Model file for the job. Use its own axes, mm. Face numbers are marked on the shaded views. A direction names the side the tool comes from. Coordinates: 2 decimals unless noted, no trailing zeros. Order: outer loops, then holes, each group sorted by start corner. A loop starts at its lowest first (then second) coordinate and runs counter-clockwise, first axis right, second up. Notation, with made-up numbers: (-14.5, 56.25) -> (35.5, 56.25) arc R19 ccw to (35.5, 72.25) -> close; hole circle Ø6 at (15, 29.5). An arc over 180 degrees is marked (long way). Return JSON: item names as keys, results as strings. Group by question number.
1) Cut at A-A (x = 0). Write the cut outline in (y, z), and give its area (3 significant figures).
2) Pull direction Y, two halves, no side cores. Call the marked faces 3 and 4: +Y half, -Y half, draft (parallel to the pull), parting line (faces both ways), or undercut.
3) Probe line 1 (Y direction, x = 0, z = 2.75); line 2 (Y direction, x = 0, z = 7.2); line 3 (X direction, y = -3.5, z = -7). List the from-to ranges inside material, lowest first.
4) Cut at C-C (z = -5). Write the cut outline in (x, y), and give its area (3 significant figures).
5) Which spindle directions (+Z, -Z, +X, -X, +Y, -Y) get a long thin tool onto all of the face, cutting with end or side? Do the marked faces 1 and 2. Say none if no direction does.
6) Flat gauge pins, fed straight in: pin 1 (4 mm diameter, centred on y = -4, z = -5.5, fed in from -X); pin 2 (1.5 mm diameter, centred on y = 3.5, z = 2.5, fed in from -X). Where does each tip first touch, or does it go through?
from build123d import *

# Parameters (mm, degrees)
SKETCH1_R           = 6
SKETCH1_R_2         = 4
BOSS_EXTRUDE1_DEPTH = 9
SKETCH2_R           = 5
CUT_EXTRUDE1_DEPTH  = 3
CHAMFER1_SIZE       = 0.2


with BuildPart() as part:
    # Sketch1 → Boss-Extrude1 (new, symmetric)
    with BuildSketch(Plane.XY):
        Circle(SKETCH1_R)
        Circle(SKETCH1_R_2, mode=Mode.SUBTRACT)
    extrude(amount=BOSS_EXTRUDE1_DEPTH, both=True)

    # Sketch2 → Cut-Extrude1 (cut)
    with BuildSketch(Plane.XY.offset(9)):
        Circle(SKETCH2_R)
    cut_extrude1 = extrude(amount=-CUT_EXTRUDE1_DEPTH, mode=Mode.SUBTRACT)

    # Mirror1: Cut-Extrude1 across plane
    add(cut_extrude1.mirror(Plane.XY), mode=Mode.SUBTRACT)

    # Chamfer1
    chamfer1_edges = [part.edges().sort_by_distance(p)[0] for p in [
        (-6, 0, -9),
        (-6, 0, 9),
    ]]
    chamfer(chamfer1_edges, length=CHAMFER1_SIZE)


solid = part.part
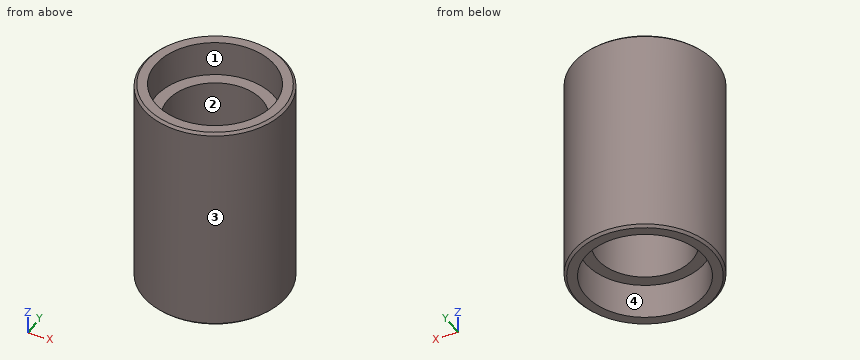
Answers below:
{
 "1": {"outline": "(-6, -8.8) -> (-5.8, -9) -> (-5, -9) -> (-5, -6) -> (-4, -6) -> (-4, 6) -> (-5, 6) -> (-5, 9) -> (-5.8, 9) -> (-6, 8.8) -> close; (4, -6) -> (5, -6) -> (5, -9) -> (5.8, -9) -> (6, -8.8) -> (6, 8.8) -> (5.8, 9) -> (5, 9) -> (5, 6) -> (4, 6) -> close", "area": "59.9 mm^2"},
 "2": {"face 3": "parting line", "face 4": "undercut"},
 "3": {"line 1": "y = -6 to -4, 4 to 6", "line 2": "y = -6 to -5, 5 to 6", "line 3": "x = -4.87 to -3.57, 3.57 to 4.87"},
 "4": {"outline": "circle Ø12 at (0, 0); hole circle Ø8 at (0, 0)", "area": "62.8 mm^2"},
 "5": {"face 1": "+Z", "face 2": "+Z, -Z"},
 "6": {"pin 1": "stops at x = -5.66", "pin 2": "stops at x = -5.33"}
}
